Work out the finished part from the listing and answer in its coordinate system (mm). A direction names the side the tool comes from. Round coordinates to 2 decimals unless told otherwise and drop trailing zeros. Write each loop counter-clockwise with the first axis right and the second up, starting at its lowest first coordinate (ties: lowest second). Pieces come first, ordered by that corner, then holes.
1. Determine the mould class of faces 3 (the face through (8, -23, -35)), 4 (the face through (-14.985, -0.66, -14.79)), 5 (the face through (12.932, -5.362, -47.255)), 6 (the face through (-23.977, -1.055, -17.745)) for opening direction X: pulls with the +X half, pulls with the -X half, needs draft (parallel to the pull), parting line crosses it, or undercut.
2. A tool of negligible diameter and unlimited length cuts with its end or side. For faces 1 (the face through (-23, 0, -45)), 2 (the face through (-10.32, 9.69, -65)), from which of +Z, -Z, +X, -X, +Y, -Y can it reach the whole face along a straight path? Write none if from no direction.
3. Flat-ended cylindrical pins translate along their axes: pin 1 Ø1 at (x, z) = (10.5, -48) entering from +Y; pin 2 Ø1.5 at (y, z) = (-1.5, -32) entering from -X; pin 3 Ø4 at (y, z) = (-5.5, -44.5) entering from -X; pin 4 Ø10 at (x, y) = (-21, 19) entering from +Z. Find the tip coordinate at first contact, or state that the pin passes through.
4. Find section D-D (z = -4). Write down the section's boundary in (x, y), and give its area (3 significant figures).
5. Find section A-A (x = 0). Write down the section's boundary in (y, z), and give its area (3 significant figures).
6. Find section C-C (z = -57). Write down the section's boundary in (x, y), and give its area (3 significant figures).
7. Straight lines are drawn through the part: probe 1 along Y at (x, z) = (0, -38); probe 2 along Y at (x, z) = (0, -50); probe 3 along Z at (x, y) = (24, -6.5). For each, find the intervals that lie inside material, in ascending order.
```python
from build123d import *

# Parameters (mm, degrees)
M30X2_0_TAPPED_HOLE1_D     = 28
M30X2_0_TAPPED_HOLE1_DEPTH = 35
M30X2_0_TAPPED_HOLE1_TIP   = 8.412048666


with BuildPart() as part:
    # Sketch1 → Revolve1 (revolve)
    with BuildSketch(Plane(origin=(0, 0, 0), x_dir=(1, 0, 0), z_dir=(0, 1, 0))):
        Polygon((15, 0), (24, 0), (24, 35), (27.5, 35), (27.5, 45), (22.5, 45), (22.5, 65), (12.5, 65), (12.5, 30), (15, 30), align=None)
    revolve(axis=Axis((0, 0, 0), (0, 0, -1)))

    # M30x2.0 Tapped Hole1
    with Locations(Plane(origin=(0, 0, -65), x_dir=(-1, 0, 0), z_dir=(0, 0, -1))):
        with Locations((0, 0)):
            Hole(M30X2_0_TAPPED_HOLE1_D / 2, depth=M30X2_0_TAPPED_HOLE1_DEPTH)
            with Locations((0, 0, -(M30X2_0_TAPPED_HOLE1_DEPTH + M30X2_0_TAPPED_HOLE1_TIP / 2))):  # 118° drill point
                Cone(0, M30X2_0_TAPPED_HOLE1_D / 2, M30X2_0_TAPPED_HOLE1_TIP, mode=Mode.SUBTRACT)


solid = part.part
```
Worked answers:
1. face 3: needs draft
1. face 4: undercut
1. face 5: undercut
1. face 6: parting line crosses it
2. face 1: -Z
2. face 2: -Z, +X, -X, +Y, -Y
3. pin 1: stops at y = 20.16
3. pin 2: stops at x = -23.99
3. pin 3: stops at x = -27.28
3. pin 4: stops at z = 0
4. outline: circle Ø48 at (0, 0); hole circle Ø30 at (0, 0)
4. area: 1,100 mm2
5. outline: (-27.5, -45) - (-22.5, -45) - (-22.5, -65) - (-14, -65) - (-14, -30) - (-15, -30) - (-15, 0) - (-24, 0) - (-24, -35) - (-27.5, -35) - close; (14, -65) - (22.5, -65) - (22.5, -45) - (27.5, -45) - (27.5, -35) - (24, -35) - (24, 0) - (15, 0) - (15, -30) - (14, -30) - close
5. area: 1,250 mm2
6. outline: circle Ø45 at (0, 0); hole circle Ø28 at (0, 0)
6. area: 975 mm2
7. probe 1: y = -27.5 to -14, 14 to 27.5
7. probe 2: y = -22.5 to -14, 14 to 22.5
7. probe 3: z = -45 to -35
